Part model, mm, in its own coordinate system. Face numbers are marked on the shaded views. A direction names the side the tool comes from. Round coordinates to 2 decimals unless told otherwise and drop trailing zeros. Loops run counter-clockwise (first coordinate to the right, second up) from the corner with the lowest first, then second, coordinate; pieces in that order, holes last.
1) Probe line 1 (Y direction, x = -7, z = 0) (3 decimals); line 2 (Y direction, x = -13.8, z = 0); line 3 (Y direction, x = 21, z = 0). List the from-to ranges inside material, lowest first.
2) 3-axis set-ups, long thin cutter, end or side, ignore diameter. For the marked faces 1, 2, 3 and 4: which of +Z, -Z, +X, -X, +Y, -Y reach the whole face in a straight line?
3) Drop flat-ended pins along their axis: P1, Ø10, axis at x = 30, y = 4.5, coming from the +Z side; P2, Ø5, axis at y = 38.5, z = 40, coming from the -X side; P3, Ø12, axis at x = -2, z = -41, coming from the +Y side. Give the stop position or say it passes through.
4) Band-saw the part on A-A, the plane x = -7. Write the cut outline in (y, z) (1 decimal).
5) Band-saw the part on B-B, the plane x = 26. Write the cut outline in (y, z), then the cut area to 3 significant figures.
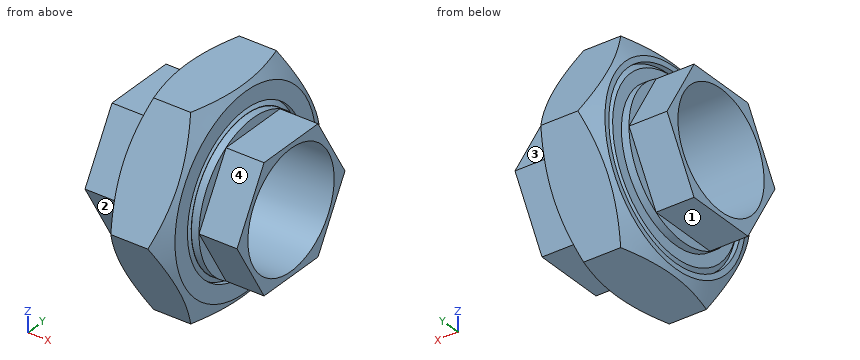
from build123d import *

# Parameters (mm, degrees)
CHAMFER_1_SIZE           = 2.606
CUT_EXTRUDE_START        = -19.5
SKETCH_4_R               = 40.3075
CUT_EXTRUDE_1_DEPTH      = 19.5
SKETCH_8_R               = 65.5435
CUT_EXTRUDE_3_DEPTH      = 101.408687124
SKETCH_10_OUTSIDE_W      = 175.022
SKETCH_10_OUTSIDE_H      = 190.988
SKETCH_10_OUTSIDE_R      = 49.0220175
CUT_EXTRUDE_4_DEPTH      = 10
CUT_EXTRUDE_4_DRAFT      = -60
MIRROR_7_COPY_1_SKETCH_W = 175.022
MIRROR_7_COPY_1_SKETCH_H = 190.988
MIRROR_7_COPY_1_SKETCH_R = 49.0220175
MIRROR_7_COPY_1_DEPTH    = 10
MIRROR_7_COPY_1_DRAFT    = -60
SKETCH_11_R              = 30
CUT_EXTRUDE_5_DEPTH      = 111.892521812
SKETCH_12_R              = 30
EXTRUDE_1_DEPTH          = 19.5
SKETCH_13_R              = 37.558920999
SKETCH_13_R_2            = 35.05
EXTRUDE_2_DEPTH          = 35.1


with BuildPart() as part:
    # 草图1 → 旋转1 (revolve)
    with BuildSketch(Plane.XY, mode=Mode.PRIVATE) as revolve_1_sk:
        Polygon((39, 35.05), (15.6, 35.05), (15.6, 40.3075), (0, 40.3075), (0, 46.266), (-15.6, 46.266), (-15.6, 35.05), (-39, 35.05), (-39, 26.877146006), (-15.6, 26.06), (15.6, 26.06), (39, 26.877146006), align=None)
    revolve(revolve_1_sk.sketch.rotate(Axis((0, 0, 0), (1, 0, 0)), 90), axis=Axis((0, 0, 0), (1, 0, 0)))

    # 倒角1
    chamfer_1_edges = [part.edges().sort_by_distance(p)[0] for p in [
        (-15.6, 0, -46.266),
        (15.6, 0, -40.3075),
    ]]
    chamfer(chamfer_1_edges, length=CHAMFER_1_SIZE)

    # 草图3 → 旋转2 (revolve)
    with BuildSketch(Plane.XY, mode=Mode.PRIVATE) as revolve_2_sk:
        Polygon((-15.6, 46.266), (-15.6, 59.585), (15.6, 59.585), (15.6, 40.3075), (0, 40.3075), (0, 46.266), align=None)
    revolve(revolve_2_sk.sketch.rotate(Axis((0, 0, 0), (1, 0, 0)), 90), axis=Axis((0, 0, 0), (1, 0, 0)))

    # 草图4 → 切除-拉伸1 (cut)
    with BuildSketch(Plane(origin=(39, 0, 0), x_dir=(0, 0, -1), z_dir=(1, 0, 0)).offset(CUT_EXTRUDE_START)):
        with Locations(Location((0, 0, 0), (0, 0, 180))):
            Circle(SKETCH_4_R)
        Polygon((0, 35.05), (-30.354190403, 17.525), (-30.354190403, -17.525), (0, -35.05), (30.354190403, -17.525), (30.354190403, 17.525), align=None, mode=Mode.SUBTRACT)
    cut_extrude_1 = extrude(amount=CUT_EXTRUDE_1_DEPTH, mode=Mode.SUBTRACT)

    # 草图6 → 旋转3 (revolve)
    with BuildSketch(Plane.XY, mode=Mode.PRIVATE) as revolve_3_sk:
        with BuildLine():
            Line((25.472011753, 26.404738247), (15.6, 26.404738247))
            Line((15.6, 26.404738247), (15.6, 36.27675))
            ThreePointArc((15.6, 36.27675), (18.491445299, 29.296183545), (25.472011753, 26.404738247))
        make_face()
    revolve_3 = revolve(revolve_3_sk.sketch.rotate(Axis((0, 0, 0), (1, 0, 0)), 120), axis=Axis((0, 0, 0), (1, 0, 0)))

    # 草图8 → 切除-拉伸3 (cut, through all)
    with BuildSketch(Plane(origin=(15.6, 0, 0), x_dir=(0, 0, -1), z_dir=(1, 0, 0))):
        Circle(SKETCH_8_R)
        Polygon((0, 59.585), (-51.602123684, 29.7925), (-51.602123684, -29.7925), (0, -59.585), (51.602123684, -29.7925), (51.602123684, 29.7925), align=None, mode=Mode.SUBTRACT)
    extrude(amount=-CUT_EXTRUDE_3_DEPTH, mode=Mode.SUBTRACT)


with BuildPart() as cut_extrude_4_tool:
    # 草图10 outside → 切除-拉伸4 (with draft: the straight prism first)
    with BuildSketch(Plane(origin=(15.6, 0, 0), x_dir=(0, 0, -1), z_dir=(1, 0, 0))):
        Rectangle(SKETCH_10_OUTSIDE_W, SKETCH_10_OUTSIDE_H)
        Circle(SKETCH_10_OUTSIDE_R, mode=Mode.SUBTRACT)
    extrude(amount=-CUT_EXTRUDE_4_DEPTH)
    # 切除-拉伸4: the draft: its side faces are tilted about the plane it starts from
    cut_extrude_4_sides = [cut_extrude_4_tool.faces().sort_by_distance(p)[0] for p in [
        (10.6, -95.494, 0),
        (10.6, 0, -87.511),
        (10.6, 95.494, 0),
        (10.6, 0, 87.511),
        (10.6, 0, 49.0220175),
    ]]
    draft(cut_extrude_4_sides, Plane(origin=(15.6, 0, 0), x_dir=(0, 0, -1), z_dir=(1, 0, 0)), CUT_EXTRUDE_4_DRAFT)


with BuildPart() as part_1:
    add(part.part)

    # 切除-拉伸4: cut by cut_extrude_4_tool
    add(cut_extrude_4_tool.part, mode=Mode.SUBTRACT)

    # 镜向7: 切除-拉伸1, 旋转3 across plane
    add(cut_extrude_1.mirror(Plane(origin=(0, 0, 0), x_dir=(0, 0, 1), z_dir=(1, 0, 0))), mode=Mode.SUBTRACT)
    add(revolve_3.mirror(Plane(origin=(0, 0, 0), x_dir=(0, 0, 1), z_dir=(1, 0, 0))))


with BuildPart() as mirror_7_copy_1_tool:
    # 镜向7 copy 1 sketch → 镜向7 copy 1 (with draft: the straight prism first)
    with BuildSketch(Plane(origin=(-15.6, 0, 0), x_dir=(0, 0, -1), z_dir=(-1, 0, 0))):
        Rectangle(MIRROR_7_COPY_1_SKETCH_W, MIRROR_7_COPY_1_SKETCH_H)
        Circle(MIRROR_7_COPY_1_SKETCH_R, mode=Mode.SUBTRACT)
    extrude(amount=-MIRROR_7_COPY_1_DEPTH)
    # 镜向7 copy 1: the draft: its side faces are tilted about the plane it starts from
    mirror_7_copy_1_sides = [mirror_7_copy_1_tool.faces().sort_by_distance(p)[0] for p in [
        (-10.6, -95.494, 0),
        (-10.6, 0, -87.511),
        (-10.6, 95.494, 0),
        (-10.6, 0, 87.511),
        (-10.6, 0, 49.0220175),
    ]]
    draft(mirror_7_copy_1_sides, Plane(origin=(-15.6, 0, 0), x_dir=(0, 0, -1), z_dir=(-1, 0, 0)), MIRROR_7_COPY_1_DRAFT)


with BuildPart() as part_2:
    add(part_1.part)

    # 镜向7 copy 1: cut by mirror_7_copy_1_tool
    add(mirror_7_copy_1_tool.part, mode=Mode.SUBTRACT)

    # 草图11 → 切除-拉伸5 (cut, through all)
    with BuildSketch(Plane.ZY.offset(39)):
        Circle(SKETCH_11_R)
    extrude(amount=-CUT_EXTRUDE_5_DEPTH, mode=Mode.SUBTRACT)

    # 草图12 → 凸台-拉伸1 (add)
    with BuildSketch(Plane.ZY.offset(39)):
        Polygon((0, 37.527767497), (-32.5, 18.763883749), (-32.5, -18.763883749), (0, -37.527767497), (32.5, -18.763883749), (32.5, 18.763883749), align=None)
        Circle(SKETCH_12_R, mode=Mode.SUBTRACT)
    extrude_1 = extrude(amount=-EXTRUDE_1_DEPTH)

    # 草图13 → 凸台-拉伸2 (add)
    with BuildSketch(Plane.ZY.offset(19.5)):
        Circle(SKETCH_13_R)
        with Locations(Location((0, 0, 0), (0, 0, 330))):
            Circle(SKETCH_13_R_2, mode=Mode.SUBTRACT)
    extrude_2 = extrude(amount=-EXTRUDE_2_DEPTH)

    # 镜向8: 凸台-拉伸1, 凸台-拉伸2 across plane
    add(extrude_1.mirror(Plane(origin=(0, 0, 0), x_dir=(0, 0, 1), z_dir=(1, 0, 0))))
    add(extrude_2.mirror(Plane(origin=(0, 0, 0), x_dir=(0, 0, 1), z_dir=(1, 0, 0))))


solid = part_2.part
Reported:
1. line 1: y = -59.585 to -30, 30 to 59.585
1. line 2: y = -52.14 to -46.27, -45.46 to -30, 30 to 45.46, 46.27 to 52.14
1. line 3: y = -37.53 to -30, 30 to 37.53
2. face 1: -Z, -X, +Y, -Y
2. face 2: -Z, -X, -Y
2. face 3: +Z, +X, +Y
2. face 4: +Z, +X, -Y
3. P1: stops at z = 32.5
3. P2: stops at x = -13.29
3. P3: stops at y = 39.38
4. outline: (-59.6, 0) - (-29.8, -51.6) - (29.8, -51.6) - (59.6, 0) - (29.8, 51.6) - (-29.8, 51.6) - close; hole circle Ø60 at (0, 0)
5. outline: (-37.53, 0) - (-18.76, -32.5) - (18.76, -32.5) - (37.53, 0) - (18.76, 32.5) - (-18.76, 32.5) - close; hole circle Ø60 at (0, 0)
5. area: 832 mm2
